Design review of the part built by this model. Coordinates are the model's own, in mm. Coordinates: 2 decimals unless noted, no trailing zeros. Write each loop counter-clockwise with the first axis right and the second up, starting at its lowest first coordinate (ties: lowest second). Pieces come first, ordered by that corner, then holes. Notation, with made-up numbers: (58.25, -25) - (116.25, -25) arc R28 ccw to (116.25, 13) - close; hole circle Ø4 at (65, -25). An arc over 180 degrees is marked (long way). Use a Markdown table: item, result.
from build123d import *

# Parameters (mm, degrees)
SKETCH_1_W               = 100
SKETCH_1_H               = 138
EXTRUDE_1_DEPTH          = 10
HOLE_WIZARD_9_0_9_1_D    = 9
SKETCH_4_R               = 22.5
CUT_EXTRUDE_1_DEPTH      = 10
HOLE_WIZARD_9_0_9_2_D    = 9
PATTERN_CIRCULAR_1_COUNT = 4
CHAMFER_1_SIZE           = 10


with BuildPart() as part:
    # 草图1 → 凸台-拉伸1 (new body)
    with BuildSketch(Plane(origin=(0, 0, 0), x_dir=(0, 0, -1), z_dir=(1, 0, 0))):
        Rectangle(SKETCH_1_W, SKETCH_1_H)
    extrude(amount=EXTRUDE_1_DEPTH)

    # Ø9.0 (9) 直径孔1 (through all)
    with Locations(Plane(origin=(10, 0, 0), x_dir=(0, 0, -1), z_dir=(1, 0, 0))):
        with Locations((-30, 44), (0, 44), (30, 44)):
            Hole(HOLE_WIZARD_9_0_9_1_D / 2)

    # 草图4 → 切除-拉伸1 (cut)
    with BuildSketch(Plane(origin=(10, 0, 0), x_dir=(0, 0, -1), z_dir=(1, 0, 0))):
        with Locations((0, -30)):
            Circle(SKETCH_4_R)
    extrude(amount=-CUT_EXTRUDE_1_DEPTH, mode=Mode.SUBTRACT)

    # Ø9.0 (9) 直径孔2 (through all)
    with Locations(Plane(origin=(10, 0, 0), x_dir=(0, 0, -1), z_dir=(1, 0, 0))):
        with Locations((-28.25, -1.75)):
            hole_wizard_9_0_9_2 = Hole(HOLE_WIZARD_9_0_9_2_D / 2)

    # 阵列(圆周)1: Ø9.0 (9) 直径孔2 ×4 about axis
    pattern_circular_1_axis = Axis((0, -30, 0), (1, 0, 0))
    for i in range(1, PATTERN_CIRCULAR_1_COUNT):
        add(hole_wizard_9_0_9_2.rotate(pattern_circular_1_axis, i * 360 / PATTERN_CIRCULAR_1_COUNT), mode=Mode.SUBTRACT)

    # 倒角1
    chamfer_1_edges = [part.edges().sort_by_distance(p)[0] for p in [
        (5, -69, -50),
        (5, -69, 50),
        (5, 69, 50),
        (5, 69, -50),
    ]]
    chamfer(chamfer_1_edges, length=CHAMFER_1_SIZE)


solid = part.part
(1) Take a section at A-A on z = 0. Write out the cut boundary in (x, y).
Determined:
| item | result |
|---|---|
| outline | (0, -69) - (10, -69) - (10, -52.5) - (0, -52.5) - close; (0, -7.5) - (10, -7.5) - (10, 39.5) - (0, 39.5) - close; (0, 48.5) - (10, 48.5) - (10, 69) - (0, 69) - close |
(2) Take a section at D-D on y = -20. Write out the cut boundary in (x, z), and give its area (3 significant figures).
Determined:
| item | result |
|---|---|
| outline | (0, -50) - (10, -50) - (10, -20.16) - (0, -20.16) - close; (0, 20.16) - (10, 20.16) - (10, 50) - (0, 50) - close |
| area | 597 mm2 |
(3) Take a section at B-B on x = 2.5. State how many separate pieces and enclosed holes the cut face has, and give its area (3 significant figures).
Determined:
| item | result |
|---|---|
| separate pieces | 1 |
| enclosed holes | 8 |
| area | 11,600 mm2 |
(4) For L1, parallel to Z at x = 1.25, y = -58; L2, parallel to Y at x = 3.75, z = 0; L3, parallel to Z at x = 7, y = 45.5, list the stretches that pass through material, from the lowest coordinate up. Write a range as from..to.
Determined:
| item | result |
|---|---|
| L1 | -50..-32.74, -23.76..23.76, 32.74..50 |
| L2 | -69..-52.5, -7.5..39.5, 48.5..69 |
| L3 | -50..-34.24, -25.76..-4.24, 4.24..25.76, 34.24..50 |
(5) Draft analysis for pull direction Y (two halves, no side actions). For faces 1 (the cylindrical face through (4.93, -0.398, 32.542)), 2 (the flat face through (5, 69, 1)), 3 (the flat face through (10, 1, 1)), state which applies: +Y half, -Y half, draft (parallel to the pull), parting line (faces both ways), or undercut.
Determined:
| item | result |
|---|---|
| face 1 | undercut |
| face 2 | +Y half |
| face 3 | draft |
(6) Take a section at C-C on z = -30. Write out the cut boundary in (x, y), and give its area (3 significant figures).
Determined:
| item | result |
|---|---|
| outline | (0, -69) - (10, -69) - (10, -62.4) - (0, -62.4) - close; (0, -54.1) - (10, -54.1) - (10, -5.9) - (0, -5.9) - close; (0, 2.4) - (10, 2.4) - (10, 39.5) - (0, 39.5) - close; (0, 48.5) - (10, 48.5) - (10, 69) - (0, 69) - close |
| area | 1,120 mm2 |
(7) For pin 1 (8 mm diameter, centred on y = -1.75, z = -28.25, fed in from -X) (3 decimals); pin 2 (5 mm diameter, centred on y = -12, z = 32, fed in from -X), all flat-tipped, find the tip position at first contact; note any pin that passes through.
Determined:
| item | result |
|---|---|
| pin 1 | through |
| pin 2 | x = 0 |
